Input: part model. Units: mm. Frame: model coordinates. A direction names the side the tool comes from. Give positions to 0.01 mm unless a question says otherwise; leave off trailing zeros. Answer as CSV lines item,"result".
```python
from build123d import *


with BuildPart() as part:
    # Sketch1 → Revolve1 (revolve)
    with BuildSketch(Plane.XY):
        with BuildLine():
            Line((-130.8, 157.5), (-151.8, 157.5))
            Line((-151.8, 157.5), (-151.8, 145.5))
            Line((-151.8, 145.5), (-151.8, 141.5))
            Line((-151.8, 141.5), (-150.8, 141.5))
            ThreePointArc((-150.8, 141.5), (-150.092893219, 141.207106781), (-149.8, 140.5))
            Line((-149.8, 140.5), (-149.8, 131.984995497))
            ThreePointArc((-149.8, 131.984995497), (-149.701421663, 131.552053256), (-149.425122031, 131.204468466))
            ThreePointArc((-149.425122031, 131.204468466), (-140.856955291, 120.42571931), (-137.8, 107))
            Line((-137.8, 107), (-137.8, 82.5))
            Line((-137.8, 82.5), (-137.8, 25))
            Line((-137.8, 25), (-144.3, 25))
            ThreePointArc((-144.3, 25), (-146.421320344, 24.121320344), (-147.3, 22))
            Line((-147.3, 22), (-147.3, 19))
            Line((-147.3, 19), (-111.3, 19))
            Line((-111.3, 19), (-111.3, 22))
            ThreePointArc((-111.3, 22), (-112.178679656, 24.121320344), (-114.3, 25))
            Line((-114.3, 25), (-125.8, 25))
            Line((-125.8, 25), (-125.8, 82.5))
            Line((-125.8, 82.5), (-125.8, 140))
            Line((-125.8, 140), (-128.3, 140))
            ThreePointArc((-128.3, 140), (-130.067766953, 140.732233047), (-130.8, 142.5))
            Line((-130.8, 142.5), (-130.8, 157.5))
        make_face()
    revolve(axis=Axis((-55, 0, 0), (-1, 0, 0)))


solid = part.part
```
Item 1: Ray query, line 1 (Z direction, x = -151.15, y = 0); line 2 (Y direction, x = -120, z = 0). Return the intervals inside material, ascending. Write a range as from..to.
The answers:
line 1,"-157.5..-141.5, 141.5..157.5"
line 2,"-25..-19, 19..25"
Item 2: Contact query for flat-ended pins moving along their axis: pin 1 (8 mm diameter, centred on y = 69, z = 32.5, fed in from -X); pin 2 (10 mm diameter, centred on y = -17.5, z = -111.5, fed in from +X); pin 3 (1 mm diameter, centred on y = -113, z = 75.5, fed in from -X). Output: stop coordinate, or through.
The answers:
pin 1,"x = -137.8"
pin 2,"x = -125.8"
pin 3,"x = -149.8"
Item 3: Mould query, pull axis Y, two halves, no side actions, for faces 1 (the face through (-125.8, 2, 29)), 2 (the face through (-149.8, 41, -126)), 3 (the face through (-127.07, -111.1, 85.19)). Classes: +Y half, -Y half, draft (parallel to the pull), parting line (faces both ways), or undercut.
The answers:
face 1,"draft"
face 2,"undercut"
face 3,"parting line"
Item 4: Reachability of faces 4 (the face through (-141.096, 23.846, -7.509)), 5 (the face through (-111.3, 7, -18)), 6 (the face through (-120.13, 23.846, -7.509)) from +Z, -Z, +X, -X, +Y, -Y: full face, straight path, thin tool, end or side. Return the list, or none.
The answers:
face 4,"-X"
face 5,"+Z, -Z, +X, +Y, -Y"
face 6,"+X"
